from build123d import *

# Parameters (mm, degrees)
SKETCH1_W           = 40
SKETCH1_H           = 180
SKETCH1_R           = 11
BOSS_EXTRUDE1_DEPTH = 16
SKETCH2_R           = 22
BOSS_EXTRUDE2_DEPTH = 20
FILLET1_R           = 5


with BuildPart() as part:
    # Sketch1 → Boss-Extrude1 (new body)
    with BuildSketch(Plane(origin=(0, 0, 0), x_dir=(1, 0, 0), z_dir=(0, 1, 0))):
        Rectangle(SKETCH1_W, SKETCH1_H)
        with Locations(Location((0, 70, 0), (0, 0, 270))):
            Circle(SKETCH1_R, mode=Mode.SUBTRACT)
        with Locations(Location((0, -70, 0), (0, 0, 90))):
            Circle(SKETCH1_R, mode=Mode.SUBTRACT)
    extrude(amount=BOSS_EXTRUDE1_DEPTH)

    # Sketch2 → Boss-Extrude2 (add, symmetric)
    with BuildSketch(Plane(origin=(0, 0, 0), x_dir=(0, 0, -1), z_dir=(1, 0, 0))):
        with BuildLine():
            Line((-42.5, 67), (-42.5, 16))
            Line((-42.5, 16), (42.5, 16))
            Line((42.5, 16), (42.5, 67))
            ThreePointArc((42.5, 67), (0, 109.5), (-42.5, 67))
        make_face()
        with Locations((0, 67)):
            Circle(SKETCH2_R, mode=Mode.SUBTRACT)
    extrude(amount=BOSS_EXTRUDE2_DEPTH, both=True)

    # Fillet1
    fillet1_edges = [part.edges().sort_by_distance(p)[0] for p in [
        (0, 16, 42.5),
        (20, 8, 90),
        (-20, 8, 90),
        (20, 8, -90),
        (-20, 8, -90),
        (0, 16, -42.5),
    ]]
    fillet(fillet1_edges, radius=FILLET1_R)


solid = part.part
The listing builds one solid part. Answer for the finished solid, in the listing's coordinates (mm). A direction names the side the tool comes from. Round coordinates to 2 decimals unless told otherwise and drop trailing zeros. Loops run counter-clockwise (first coordinate to the right, second up) from the corner with the lowest first, then second, coordinate; pieces in that order, holes last. Notation, with made-up numbers: M 67,11 L 76,11 A27 cw 76,38 Z; hole C 38,29.25 d10. An arc over 180 degrees is marked long. Write each question's results on one line, items separated by ' | '. Start each with the question number.
1) Determine the mould class of faces 1 (the cylindrical face through (0, 8, 81)), 2 (the flat face through (0, 0, -1)), 3 (the flat face through (-20, 42, 1)), 4 (the cylindrical face through (0, 8, -81)) for opening direction X: pulls with the +X half, pulls with the -X half, needs draft (parallel to the pull), parting line crosses it, or undercut.
2) Find section D-D on x = -8. Write down the section's boundary in (y, z), plus the area to 3 significant figures.
3) Find section C-C on y = 51. Write down the section's boundary in (x, z).
4) Each of these flat-tipped pins is pushed along its axis until it touches: pin 1 (1 mm diameter, centred on x = 12, z = -62, fed in from +Y); pin 2 (8 mm diameter, centred on x = -10.5, y = 96.5, fed in from +Z); pin 3 (20 mm diameter, centred on x = -2, y = 34, fed in from -Z); pin 4 (10 mm diameter, centred on x = 8.5, z = 11, fed in from -Y). Where does it stop, or does it pass through?
5) Straight lines are drawn through the part: probe 1 along X at (y, z) = (9, -70); probe 2 along Y at (x, z) = (12, 0.5); probe 3 along Z at (x, y) = (-13.5, 30.5). For each, find the intervals that lie inside material, in ascending order.
6) Which of the six approach directions +Z, -Z, +X, -X, +Y, -Y give full straight-line access (tool end or side, diameter ignored) to faces 5 (the flat face through (0, 44, 42.5)), 6 (the cylindrical face through (-0.28, 81.869, 16.215)), 7 (the flat face through (0, 44, -42.5))?
7) Find section A-A on x = 0. Write down the section's boundary in (y, z), plus the area to 3 significant figures.
8) Find section B-B on z = 0. Write down the section's boundary in (x, y).
Final values:
1) face 1: undercut | face 2: needs draft | face 3: pulls with the -X half | face 4: undercut
2) outline: M 0,-90 L 16,-90 L 16,-77.55 L 0,-77.55 Z; M 0,-62.45 L 16,-62.45 L 16,-47.5 A5 cw 21,-42.5 L 67,-42.5 A42.5 ccw 67,42.5 L 21,42.5 A5 cw 16,47.5 L 16,62.45 L 0,62.45 Z; M 0,77.55 L 16,77.55 L 16,90 L 0,90 Z; hole C 67,0 d44 | area: 8,060 mm²
3) outline: M -20,-42.5 L 20,-42.5 L 20,-15.1 L -20,-15.1 Z; M -20,15.1 L 20,15.1 L 20,42.5 L -20,42.5 Z
4) pin 1: y = 16 | pin 2: z = 34 | pin 3: z = -42.5 | pin 4: y = 0
5) probe 1: -20 to -11, 11 to 20 | probe 2: 0 to 45.01, 88.99 to 109.5 | probe 3: -42.5 to 42.5
6) face 5: +Z, +X, -X, +Y | face 6: +X, -X | face 7: -Z, +X, -X, +Y
7) outline: M 0,-90 L 16,-90 L 16,-81 L 0,-81 Z; M 0,-59 L 16,-59 L 16,-47.5 A5 cw 21,-42.5 L 67,-42.5 A42.5 ccw 67,42.5 L 21,42.5 A5 cw 16,47.5 L 16,59 L 0,59 Z; M 0,81 L 16,81 L 16,90 L 0,90 Z; hole C 67,0 d44 | area: 7,840 mm²
8) outline: M -20,0 L 20,0 L 20,45 L -20,45 Z; M -20,89 L 20,89 L 20,109.5 L -20,109.5 Z
